The model under review builds one solid part; all positions refer to its coordinate system, in mm. A direction names the side the tool comes from. Give positions to 0.01 mm unless a question says otherwise; leave off trailing zeros. Order: outer loops, then holes, each group sorted by start corner. A loop starts at its lowest first (then second) coordinate and runs counter-clockwise, first axis right, second up. Notation, with made-up numbers: (27, -9.5) - (58, -9.5) arc R21 ccw to (58, 23.5) - close; hole circle Ø3 at (48, -31). An arc over 180 degrees is marked (long way). Use CSV: the item, a comma, the result in double quotes.
```python
from build123d import *

# Parameters (mm, degrees)
BOSS_EXTRUDE1_DEPTH = 12.5
SKETCH3_R           = 8.7
BOSS_EXTRUDE2_DEPTH = 70
BOSS_EXTRUDE3_DEPTH = 9.5
HOLE1_D             = 4.134
HOLE1_DEPTH         = 5.5
HOLE1_CSINK_D       = 5
HOLE1_CSINK_ANGLE   = 90
HOLE1_TIP           = 1.193383006
HOLE2_D             = 4.134
HOLE2_DEPTH         = 5.5
HOLE2_CSINK_D       = 5
HOLE2_CSINK_ANGLE   = 90
HOLE2_TIP           = 1.193383006


with BuildPart() as part:
    # Sketch1 → Revolve1 (revolve)
    with BuildSketch(Plane.XY, mode=Mode.PRIVATE) as revolve1_sk:
        Polygon((-8, 0), (-8, 4.3865), (-7.3865, 5), (0, 5), (0, 0), align=None)
    revolve(revolve1_sk.sketch.rotate(Axis((0, 0, 0), (-1, 0, 0)), 270), axis=Axis((0, 0, 0), (-1, 0, 0)))

    # Sketch2 → Boss-Extrude1 (add)
    with BuildSketch(Plane(origin=(0, 0, 0), x_dir=(0, 0, -1), z_dir=(1, 0, 0))):
        with BuildLine():
            Line((-4.034538387, -9.15), (4.034538387, -9.15))
            ThreePointArc((4.034538387, -9.15), (7.071067812, -7.071067812), (9.15, -4.034538387))
            Line((9.15, -4.034538387), (9.15, 4.034538387))
            ThreePointArc((9.15, 4.034538387), (7.071067812, 7.071067812), (4.034538387, 9.15))
            Line((4.034538387, 9.15), (-4.034538387, 9.15))
            ThreePointArc((-4.034538387, 9.15), (-7.071067812, 7.071067812), (-9.15, 4.034538387))
            Line((-9.15, 4.034538387), (-9.15, -4.034538387))
            ThreePointArc((-9.15, -4.034538387), (-7.071067812, -7.071067812), (-4.034538387, -9.15))
        make_face()
    extrude(amount=BOSS_EXTRUDE1_DEPTH)

    # Sketch3 → Boss-Extrude2 (add)
    with BuildSketch(Plane(origin=(12.5, 0, 0), x_dir=(0, 0, -1), z_dir=(1, 0, 0))):
        Circle(SKETCH3_R)
    extrude(amount=BOSS_EXTRUDE2_DEPTH)

    # Sketch4 → Boss-Extrude3 (add)
    with BuildSketch(Plane(origin=(82.5, 0, 0), x_dir=(0, 0, -1), z_dir=(1, 0, 0))):
        with BuildLine():
            Line((-4.034538387, -9.15), (4.034538387, -9.15))
            ThreePointArc((4.034538387, -9.15), (7.071067812, -7.071067812), (9.15, -4.034538387))
            Line((9.15, -4.034538387), (9.15, 4.034538387))
            ThreePointArc((9.15, 4.034538387), (7.071067812, 7.071067812), (4.034538387, 9.15))
            Line((4.034538387, 9.15), (-4.034538387, 9.15))
            ThreePointArc((-4.034538387, 9.15), (-7.071067812, 7.071067812), (-9.15, 4.034538387))
            Line((-9.15, 4.034538387), (-9.15, -4.034538387))
            ThreePointArc((-9.15, -4.034538387), (-7.071067812, -7.071067812), (-4.034538387, -9.15))
        make_face()
    extrude(amount=BOSS_EXTRUDE3_DEPTH)

    # Hole1
    with Locations(Plane(origin=(0, 9.15, 0), x_dir=(1, 0, 0), z_dir=(0, 1, 0))):
        with Locations((8, 0)):
            CounterSinkHole(HOLE1_D / 2, HOLE1_CSINK_D / 2, depth=HOLE1_DEPTH, counter_sink_angle=HOLE1_CSINK_ANGLE)
            with Locations((0, 0, -(HOLE1_DEPTH + HOLE1_TIP / 2))):  # 120° drill point
                Cone(0, HOLE1_D / 2, HOLE1_TIP, mode=Mode.SUBTRACT)

    # Hole2
    with Locations(Plane(origin=(0, 9.15, 0), x_dir=(1, 0, 0), z_dir=(0, 1, 0))):
        with Locations((87, 0)):
            CounterSinkHole(HOLE2_D / 2, HOLE2_CSINK_D / 2, depth=HOLE2_DEPTH, counter_sink_angle=HOLE2_CSINK_ANGLE)
            with Locations((0, 0, -(HOLE2_DEPTH + HOLE2_TIP / 2))):  # 120° drill point
                Cone(0, HOLE2_D / 2, HOLE2_TIP, mode=Mode.SUBTRACT)

    # Sketch9 → Cut-Revolve1 (revolve, cut)
    with BuildSketch(Plane.XY, mode=Mode.PRIVATE) as cut_revolve1_sk:
        Polygon((-8, 0), (-8, 2.5), (12.5, 2.5), (12.5, 8), (62.5, 8), (62.5, 0), align=None)
    revolve(cut_revolve1_sk.sketch.rotate(Axis((50, 0, 0), (-1, 0, 0)), 270), axis=Axis((50, 0, 0), (-1, 0, 0)), mode=Mode.SUBTRACT)


solid = part.part
```
Item 1: Wall thickness on L1, parallel to X at y = 4.5, z = 7.75; L2, parallel to Y at x = 39.5, z = 0; L3, parallel to Y at x = -2.75, z = 0: over which ranges is each line inside the solid? List them lowest first.
Results list:
L1,"x = 0 to 12.5, 82.5 to 92"
L2,"y = -8.7 to -8, 8 to 8.7"
L3,"y = -5 to -2.5, 2.5 to 5"
Item 2: Mouldability with a two-part tool opening along Y and no side actions: class faces 1 (the face through (37.85, -7.81, -1.73)), 2 (the face through (47.01, -8.493, 1.886)), 3 (the face through (10.065, 6.148, -0.091)) as pulls with the +Y half, pulls with the -Y half, needs draft (parallel to the pull), parting line crosses it, or undercut.
Results list:
face 1,"undercut"
face 2,"parting line crosses it"
face 3,"needs draft"
Item 3: Take a section at B-B, the plane z = 7. Give the boundary of the cut face in (x, y).
Results list:
outline,"(0, -7.14) - (12.5, -7.14) - (12.5, -5.17) - (82.5, -5.17) - (82.5, -7.14) - (92, -7.14) - (92, 7.14) - (82.5, 7.14) - (82.5, 5.17) - (12.5, 5.17) - (12.5, 7.14) - (0, 7.14) - close; hole (12.5, -3.87) - (62.5, -3.87) - (62.5, 3.87) - (12.5, 3.87) - close"
Item 4: Take a section at C-C, the plane x = 26. Give the boundary of the cut face in (y, z), and give its area (3 significant figures).
Results list:
outline,"circle Ø17.4 at (0, 0); hole circle Ø16 at (0, 0)"
area,"36.7 mm2"
Item 5: Tool access review of faces 4 (the face through (0, -4, -4)), 5 (the face through (-8, -2, -2)), 6 (the face through (62.5, 0, 0)), 7 (the face through (85.03, 6.15, -0.62)), 8 (the face through (87.18, -7.03, 7.11)): name each direction out of +Z, -Z, +X, -X, +Y, -Y from which nothing blocks a thin tool from reaching the whole face with its end or side.
Results list:
face 4,"-X"
face 5,"+Z, -Z, -X, +Y, -Y"
face 6,"none"
face 7,"+Y"
face 8,"+Z, +X, -X, -Y"
Item 6: Clearance check with flat-ended pins moving along their axes: pin 1 (10 mm diameter, centred on x = 43.5, z = 3.5, fed in from +Y); pin 2 (1 mm diameter, centred on x = 42, y = 0.5, fed in from +Z); pin 3 (4 mm diameter, centred on x = 77, y = -6, fed in from +Z). State where each tip first meets the part, or that it passes through.
Results list:
pin 1,"stops at y = 8.7"
pin 2,"stops at z = 8.7"
pin 3,"stops at z = 7.73"
Item 7: Take a section at A-A, the plane y = 0. Give the boundary of the cut face in (x, z), and give its area (3 significant figures).
Results list:
outline,"(-8, -4.39) - (-7.39, -5) - (0, -5) - (0, -9.15) - (12.5, -9.15) - (12.5, -8.7) - (82.5, -8.7) - (82.5, -9.15) - (92, -9.15) - (92, 9.15) - (82.5, 9.15) - (82.5, 8.7) - (12.5, 8.7) - (12.5, 9.15) - (0, 9.15) - (0, 5) - (-7.39, 5) - (-8, 4.39) - (-8, 2.5) - (12.5, 2.5) - (12.5, 8) - (62.5, 8) - (62.5, -8) - (12.5, -8) - (12.5, -2.5) - (-8, -2.5) - close"
area,"798 mm2"
